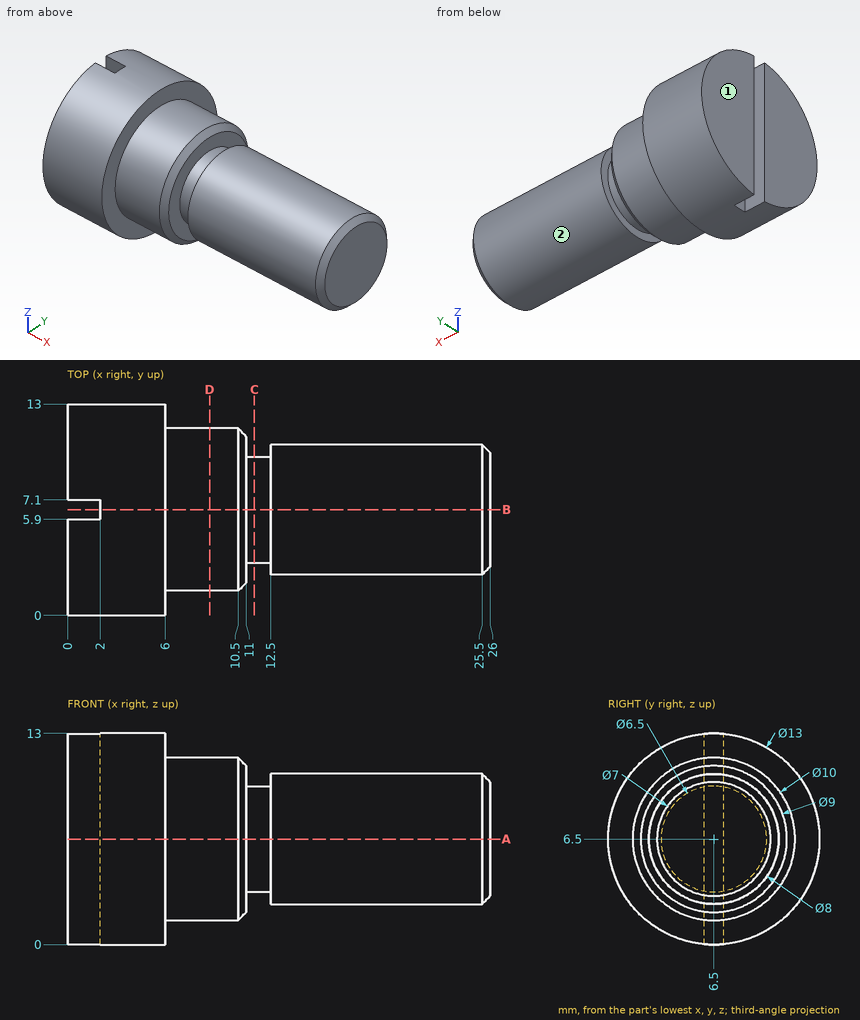
Here's the drawing with two shaded views (mm, measured from the low corner). I have some questions. A direction names the side the tool comes from. Coordinates: 2 decimals unless noted, no trailing zeros. Write each loop counter-clockwise with the first axis right and the second up, starting at its lowest first coordinate (ties: lowest second). Pieces come first, ordered by that corner, then holes. Notation, with made-up numbers: (-9, 15.25) -> (47, 15.25) arc R30 ccw to (47, 52.25) -> close; hole circle Ø7 at (-31, 72). An arc over 180 degrees is marked (long way). One line per question, with ' | ' between items. Start each with the question number.
1. If we section it at A-A (z = 6.5): Please give me the cut outline in (x, y).
2. Will these pins go through, and if not, where does the flat tip stop? P1, Ø0.6, axis at y = 6.5, z = 3.5, coming from the -X side; P2, Ø1, axis at y = 4, z = 3, coming from the -X side; P3, Ø3, axis at x = 13, z = 10.5, coming from the +Y side; P4, Ø4, axis at x = 16.5, z = 5, coming from the +Y side.
3. If we section it at C-C (x = 11.5): Please give me the cut outline in (y, z).
4. For the marked faces 1 and 2, which set-ups out of +Z, -Z, +X, -X, +Y, -Y let a thin tool reach every point of the face, with its end or its side?
5. If we section it at B-B (y = 6.5): Please give me the cut outline in (x, z), and give its area (3 significant figures).
6. If we section it at D-D (x = 8.75): Please give me the cut outline in (y, z).
7. Please list where these lines run through material, in increasing order: line 1 along X through (y, z) = (8.5, 1.75); line 2 along X through (y, z) = (5, 10.25); line 3 along Z through (x, y) = (14.5, 7).
Return value:
1) outline: (0, 0) -> (6, 0) -> (6, 1.5) -> (10.5, 1.5) -> (11, 2) -> (11, 3.25) -> (12.5, 3.25) -> (12.5, 2.5) -> (25.5, 2.5) -> (26, 3) -> (26, 10) -> (25.5, 10.5) -> (12.5, 10.5) -> (12.5, 9.75) -> (11, 9.75) -> (11, 11) -> (10.5, 11.5) -> (6, 11.5) -> (6, 13) -> (0, 13) -> (0, 7.1) -> (2, 7.1) -> (2, 5.9) -> (0, 5.9) -> close
2) P1: stops at x = 2 | P2: stops at x = 0 | P3: stops at y = 9.62 | P4: stops at y = 10.5
3) outline: circle Ø6.5 at (6.5, 6.5)
4) face 1: +Z, -Z, -X, +Y, -Y | face 2: +X
5) outline: (2, 0) -> (6, 0) -> (6, 1.5) -> (10.5, 1.5) -> (11, 2) -> (11, 3.25) -> (12.5, 3.25) -> (12.5, 2.5) -> (25.5, 2.5) -> (26, 3) -> (26, 10) -> (25.5, 10.5) -> (12.5, 10.5) -> (12.5, 9.75) -> (11, 9.75) -> (11, 11) -> (10.5, 11.5) -> (6, 11.5) -> (6, 13) -> (2, 13) -> close | area: 219 mm²
6) outline: circle Ø10 at (6.5, 6.5)
7) line 1: x = 0 to 6 | line 2: x = 0 to 11 | line 3: z = 2.53 to 10.47
